Job drawing, mm, ordinate dimensions from the low corner. One solid piece. A direction names the side the tool comes from. Coordinates: 2 decimals unless noted, no trailing zeros. Loops run counter-clockwise (first coordinate to the right, second up) from the corner with the lowest first, then second, coordinate; pieces in that order, holes last. Notation, with made-up numbers: M 30.25,85.5 L 78.25,85.5 A24 ccw 78.25,115.5 Z; hole C 84,5.25 d3. An arc over 180 degrees is marked long. Answer as a JSON object with one key per item and string values. Group by question number.
1. Drop flat-ended pins along their axis: pin 1 Ø4 at (x, y) = (15, 7.5) entering from +Z (1 decimal); pin 2 Ø3 at (x, y) = (52, 9.5) entering from -Z; pin 3 Ø4 at (x, y) = (34.5, 4) entering from +Z; pin 4 Ø6.5 at (x, z) = (27.97, 43.38) entering from -Y. Give the stop position or say it passes through.
2. Saw through at B-B on y = 15.25. Write the cut outline in (x, z).
3. 3-axis set-ups, long thin cutter, end or side, ignore diameter. For the marked faces 4 and 5: which of +Z, -Z, +X, -X, +Y, -Y reach the whole face in a straight line?
4. Mould opens along Z. For the marked faces 1, 2 and 3 say: released by +Z, released by -Z, zero draft, split by the parting line, or undercut.
5. Saw through at C-C on x = 9.5. Write the cut outline in (y, z), then the cut area to 3 significant figures.
6. Saw through at D-D on z = 72.5. Write the cut outline in (x, y), then the cut area to 3 significant figures.
7. Saw through at A-A on z = 40. Write the cut outline in (x, y) (1 decimal), then the cut area to 3 significant figures.
8. Drill centre lines: L1, parallel to X at y = 12.75, z = 43 (1 decimal); L2, parallel to X at y = 19.25, z = 38.5 (1 decimal); L3, parallel to Z at x = 41, y = 15.5. Where is each one in solid material? Low to high.
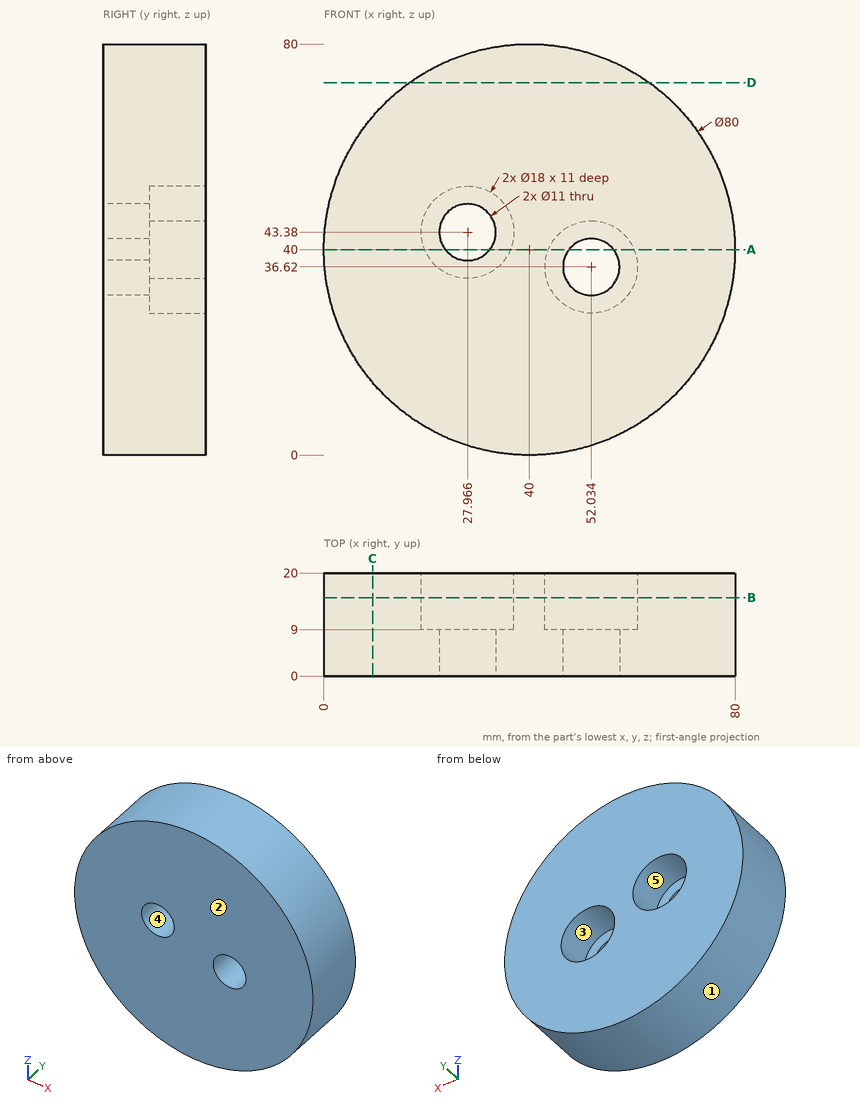
Outcome:
{
 "1": {"pin 1": "stops at z = 72.7", "pin 2": "stops at z = 1.4", "pin 3": "stops at z = 79.85", "pin 4": "passes through"},
 "2": {"outline": "C 40,40 d80; hole C 27.97,43.38 d18; hole C 52.03,36.62 d18"},
 "3": {"face 4": "+Y, -Y", "face 5": "+Y"},
 "4": {"face 1": "split by the parting line", "face 2": "zero draft", "face 3": "undercut"},
 "5": {"outline": "M 0,14.12 L 20,14.12 L 20,65.88 L 0,65.88 Z", "area": "1,040 mm²"},
 "6": {"outline": "M 16.68,0 L 63.32,0 L 63.32,20 L 16.68,20 Z", "area": "933 mm²"},
 "7": {"outline": "M 0,0 L 23.6,0 L 23.6,9 L 19.6,9 L 19.6,20 L 0,20 Z; M 32.3,0 L 47.7,0 L 47.7,9 L 43.7,9 L 43.7,20 L 36.3,20 L 36.3,9 L 32.3,9 Z; M 56.4,0 L 80,0 L 80,20 L 60.4,20 L 60.4,9 L 56.4,9 Z", "area": "1,080 mm²"},
 "8": {"L1": "x = 0.1 to 19, 37 to 45.7, 58.4 to 79.9", "L2": "x = 0 to 20.4, 35.5 to 43.2, 60.8 to 80", "L3": "z = 0.01 to 79.99"}
}
